```python
from build123d import *

# Parameters (mm, degrees)
HEX_BODY_16AF_X_11_DEPTH = 5.5
BORE_SKETCH_10_R         = 5
BORE_10_THROUGH_DEPTH    = 17.441816779


with BuildPart() as part:
    # Hex Profile 16AF Sketch → Hex Body 16AF x 11 (new, symmetric)
    with BuildSketch(Plane(origin=(0, 0, 0), x_dir=(1, 0, 0), z_dir=(0, 1, 0))):
        Polygon((9.237604307, 0), (4.618802154, 8), (-4.618802154, 8), (-9.237604307, 0), (-4.618802154, -8), (4.618802154, -8), align=None)
    extrude(amount=HEX_BODY_16AF_X_11_DEPTH, both=True)

    # Chamfer Profile Sketch → Face Chamfer 2mm (revolve, cut)
    with BuildSketch(Plane.XY, mode=Mode.PRIVATE) as face_chamfer_2mm_sk:
        with BuildLine():
            Line((9.237604307, 3.5), (9.237604307, -5.5))
            Line((9.237604307, -5.5), (12.102974232, -5.5))
            Line((12.102974232, -5.5), (12.102974232, 7.625857748))
            Line((12.102974232, 7.625857748), (4.618802154, 7.625857748))
            Line((4.618802154, 7.625857748), (4.618802154, 5.5))
            Line((4.618802154, 5.5), (7.237604307, 5.5))
            ThreePointArc((7.237604307, 5.5), (8.651817869, 4.914213562), (9.237604307, 3.5))
        make_face()
    revolve(face_chamfer_2mm_sk.sketch.rotate(Axis((0, 0, 0), (0, 1, 0)), 90), axis=Axis((0, 0, 0), (0, 1, 0)), mode=Mode.SUBTRACT)

    # Bore Sketch Ø10 → Bore Ø10 Through (cut, through all)
    with BuildSketch(Plane(origin=(0, 5.5, 0), x_dir=(1, 0, 0), z_dir=(0, 1, 0))):
        with Locations(Location((0, 0, 0), (0, 0, 270))):
            Circle(BORE_SKETCH_10_R)
    extrude(amount=-BORE_10_THROUGH_DEPTH, mode=Mode.SUBTRACT)


solid = part.part
```
The model under review builds one solid part; all positions refer to its coordinate system, in mm. Give positions to 0.01 mm unless a question says otherwise; leave off trailing zeros. Write each loop counter-clockwise with the first axis right and the second up, starting at its lowest first coordinate (ties: lowest second). Pieces come first, ordered by that corner, then holes.
(1) The part is to be moulded in two halves that separate along X. For faces 1 (the flat face through (6.896, 0, 4.056)), 2 (the flat face through (5, 5.5, -2)), 3 (the cylindrical face through (-4.88, 0.08, -1.08)), 4 (the flat face through (-6.961, 0, 3.944)), say which applies: released by +X, released by -X, zero draft, split by the parting line, or undercut.
(2) Consider section C-C, the plane y = 4. Give the boundary of the cut face in (x, z).
(3) Consider section A-A, the plane x = 0. Give the boundary of the cut face in (y, z).
(4) For P1, Ø1, axis at y = -4.5, z = 3, coming from the -X side; P2, Ø8, axis at x = 0, z = 0, coming from the -Y side; P3, Ø1, axis at x = -6, y = -2.5, coming from the -Z side; P4, Ø1.5, axis at y = 2, z = -4, coming from the +X side, all flat-tipped, find the tip position at first contact; note any pin that passes through.
(5) Consider section B-B, the plane y = -3. Give the boundary of the cut face in (x, z), and give its area (3 significant figures).
(6) To check wall thickness, follow L1, parallel to Z at x = 1, y = 1; L2, parallel to Z at x = -0.5, y = 2; L3, parallel to X at y = 3.75, z = 0. State the ranges of each line that lie inside material, in increasing order.
Returned:
1. face 1: released by +X
1. face 2: zero draft
1. face 3: undercut
1. face 4: released by -X
2. outline: (-9.17, -0.11) - (-4.68, -7.89) arc R9.17 ccw to (-4.49, -8) - (4.49, -8) arc R9.17 ccw to (4.68, -7.89) - (9.17, -0.11) arc R9.17 ccw to (9.17, 0.11) - (4.68, 7.89) arc R9.17 ccw to (4.49, 8) - (-4.49, 8) arc R9.17 ccw to (-4.68, 7.89) - (-9.17, 0.11) arc R9.17 ccw to start; hole circle Ø10 at (0, 0)
3. outline: (-5.5, -8) - (5.35, -8) arc R2 ccw to (5.5, -7.24) - (5.5, -5) - (-5.5, -5) - close; (-5.5, 5) - (5.5, 5) - (5.5, 7.24) arc R2 ccw to (5.35, 8) - (-5.5, 8) - close
4. P1: stops at x = -7.79
4. P2: passes through
4. P3: stops at z = -6.47
4. P4: stops at x = 7.36
5. outline: (-9.24, 0) - (-4.62, -8) - (4.62, -8) - (9.24, 0) - (4.62, 8) - (-4.62, 8) - close; hole circle Ø10 at (0, 0)
5. area: 143 mm2
6. L1: z = -8 to -4.9, 4.9 to 8
6. L2: z = -8 to -4.97, 4.97 to 8
6. L3: x = -9.22 to -5, 5 to 9.22
